```python
from build123d import *

# Parameters (mm, degrees)
CUT_EXTRUDE_1_DEPTH = 4
CUT_EXTRUDE_START   = -1.3
SKETCH_3_R          = 15
SKETCH_3_R_2        = 14.3
CUT_EXTRUDE_2_DEPTH = 1.3


with BuildPart() as part:
    # 草图1 → 旋转1 (revolve)
    with BuildSketch(Plane.XY, mode=Mode.PRIVATE) as revolve_1_sk:
        Polygon((0, 0), (0, 15), (43, 15), (43, 17.5), (223, 17.5), (223, 25), (233, 25), (233, 60), (1083, 60), (1083, 25), (1093, 25), (1093, 17.5), (1221, 17.5), (1221, 0), align=None)
    revolve(revolve_1_sk.sketch.rotate(Axis((0, 0, 0), (1, 0, 0)), 90), axis=Axis((0, 0, 0), (1, 0, 0)))

    # 草图2 → 切除-拉伸1 (cut)
    with BuildSketch(Plane(origin=(0, 15, 0), x_dir=(1, 0, 0), z_dir=(0, 1, 0))):
        with BuildLine():
            Line((33, 4), (-10, 4))
            Line((-10, 4), (-10, -4))
            Line((-10, -4), (33, -4))
            ThreePointArc((33, -4), (37, 0), (33, 4))
        make_face()
    extrude(amount=-CUT_EXTRUDE_1_DEPTH, mode=Mode.SUBTRACT)

    # 草图3 → 切除-拉伸2 (cut)
    with BuildSketch(Plane.ZY.offset(-9.8).offset(CUT_EXTRUDE_START)):
        Circle(SKETCH_3_R)
        Circle(SKETCH_3_R_2, mode=Mode.SUBTRACT)
    extrude(amount=CUT_EXTRUDE_2_DEPTH, mode=Mode.SUBTRACT)


solid = part.part
```
Input: part model. Units: mm. Frame: model coordinates. A direction names the side the tool comes from. Coordinates: 2 decimals unless noted, no trailing zeros. Loops run counter-clockwise (first coordinate to the right, second up) from the corner with the lowest first, then second, coordinate; pieces in that order, holes last. Notation, with made-up numbers: (12.5, 71.5) -> (53.5, 71.5) arc R25 cw to (53.5, 95.5) -> close; hole circle Ø11 at (25.5, -21.75). An arc over 180 degrees is marked (long way). Use a Markdown table: item, result.
1) Cut plane B-B (x = 733). Return the cut outline in (y, z), then the cut area to 3 significant figures.
Results found:
| item | result |
|---|---|
| outline | circle Ø120 at (0, 0) |
| area | 11,300 mm2 |
2) Material intervals for line 1 along X through (y, z) = (11.5, 42); line 2 along X through (y, z) = (-22, -9); line 3 along Y through (x, z) = (805, -5), sorted ascending. Write a range as from..to.
Results found:
| item | result |
|---|---|
| line 1 | x = 233..1083 |
| line 2 | x = 223..1093 |
| line 3 | y = -59.79..59.79 |
3) Contact query for flat-ended pins moving along their axis: pin 1 (8 mm diameter, centred on x = 127.5, z = -12, fed in from -Y); pin 2 (10 mm diameter, centred on x = 272, z = -43, fed in from -Y); pin 3 (6.5 mm diameter, centred on x = 23, z = 0.5, fed in from +Y). Output: stop coordinate, or through.
Results found:
| item | result |
|---|---|
| pin 1 | stops at y = -15.56 |
| pin 2 | stops at y = -46.43 |
| pin 3 | stops at y = 11 |
4) Access query for faces 1 (the flat face through (11.1, -14.4, 2.2)), 2 (the cylindrical face through (1088.07, -7.509, 23.846)), 3 (the flat face through (0, 0, 0)). Directions: +Z, -Z, +X, -X, +Y, -Y. A direction counts if a zero-diameter tool reaches every point of the face in a straight line with its end or side. Return the directions, or none.
Results found:
| item | result |
|---|---|
| face 1 | none |
| face 2 | +X |
| face 3 | +Z, -Z, -X, +Y, -Y |
